Here's how the part is built. I have some questions about the finished solid (model axes, mm). A direction names the side the tool comes from. Round coordinates to 2 decimals unless told otherwise and drop trailing zeros. Loops run counter-clockwise (first coordinate to the right, second up) from the corner with the lowest first, then second, coordinate; pieces in that order, holes last. Notation, with made-up numbers: (85, 16) - (126, 16) arc R17 ccw to (126, 49) - close; hole circle Ø5 at (-21, -28.5). An arc over 180 degrees is marked (long way). Answer as a JSON object with one key per item and string values. Group by question number.
1) If I drill on line 1 along X through (y, z) = (43, 50); line 2 along X through (y, z) = (-6, 59.5); line 3 along Y through (x, z) = (5, 32), over which ranges is the centre line in solid material (lowest first)? Write a range as [from, to].
2) I want a section at A-A, the plane z = 32. Please give me the cut outline in (x, y), then the cut area to 3 significant figures.
3) If we mould it in two halves opening along X, with no side actions, what happens to faces 5 (the face through (-25, 38, 32)), 6 (the face through (-50, 2, 63)), 7 (the face through (12.082, 85.524, 27.664))? For each: pulls with the +X half, pulls with the -X half, needs draft (parallel to the pull), parting line crosses it, or undercut.
4) I want a section at D-D, the plane y = 2. Please give me the cut outline in (x, z), then the cut area to 3 significant figures.
5) I want a section at C-C, the plane y = 79. Please give me the cut outline in (x, z), then the cut area to 3 significant figures.
6) Which directions (+Z, -Z, +X, -X, +Y, -Y) give clear straight access to the entire face, cutting with the end or side of a thin tool? Please do faces 1 (the face through (37, 24, 30)), 2 (the face through (-57.098, 27.468, 58.084)), 3 (the face through (28, 21, 35)), 4 (the face through (-37, -6, 32)).
7) I want a section at B-B, the plane x = 6. Please give me the cut outline in (y, z), then the cut area to 3 significant figures.
8) Will these pins go through, and if not, where does the flat tip stop? P1, Ø8, axis at x = 4.5, z = 39, coming from the -Y side; P2, Ø10, axis at x = 9.5, y = 66.5, coming from the +Z side; P3, Ø15.5, axis at x = -15.74, z = 49.83, coming from the +Y side.
from build123d import *

# Parameters (mm, degrees)
BASE_PROFILE_SKETCH_W           = 128
BASE_PROFILE_SKETCH_H           = 20
BASE_PLATE_DEPTH                = 64
UNDERSIDE_RELIEF_CUT_DEPTH      = 92.060419503
UNDERSIDE_RELIEF_CUT_DEPTH_BACK = 64
UNDERSIDE_RELIEF_SKETCH_W       = 55
UNDERSIDE_RELIEF_SKETCH_H       = 8
FIRST_UPRIGHT_SKETCH_W          = 14
FIRST_UPRIGHT_SKETCH_H          = 64
FIRST_UPRIGHT_DEPTH             = 56
FIRST_TRUNNION_BOSS_DEPTH       = 10
FIRST_TRUNNION_BOSS_DEPTH_BACK  = 14
FIRST_TRUNNION_BOSS_SKETCH_R    = 20
FIRST_TRUNNION_BOSS_SKETCH_R_2  = 10
FIRST_TRUNNION_BORE_DEPTH       = 14
FIRST_UPRIGHT_TAPER_CUT_DEPTH   = 14
CENTER_BLOCK_DEPTH              = 28
SECOND_TRUNNION_BOSS_SKETCH_R   = 20
SECOND_TRUNNION_BOSS_SKETCH_R_2 = 10
SECOND_TRUNNION_BOSS_DEPTH      = 20
SECOND_UPRIGHT_DEPTH            = 10
SECOND_TRUNNION_BORE_DEPTH      = 10
GUSSET_RIB_REACH                = 120.44
GUSSET_RIB_SKETCH_WALL_W        = 299.707341614
GUSSET_RIB_SKETCH_WALL_H        = 10
BASE_MOUNTING_HOLES_SKETCH_R    = 6
BASE_MOUNTING_HOLES_DEPTH       = 124.887045328


with BuildPart() as part:
    # Base Profile Sketch → Base Plate (new body)
    with BuildSketch(Plane.XY):
        Rectangle(BASE_PROFILE_SKETCH_W, BASE_PROFILE_SKETCH_H)
    extrude(amount=BASE_PLATE_DEPTH)

    # Underside Relief Sketch → Underside Relief Cut (cut, two sides: drawn at the far end of the back side and taken through both)
    with BuildSketch(Plane.XY.offset(-UNDERSIDE_RELIEF_CUT_DEPTH_BACK)):
        with Locations((-9.5, -6)):
            Rectangle(UNDERSIDE_RELIEF_SKETCH_W, UNDERSIDE_RELIEF_SKETCH_H)
    extrude(amount=UNDERSIDE_RELIEF_CUT_DEPTH + UNDERSIDE_RELIEF_CUT_DEPTH_BACK, mode=Mode.SUBTRACT)

    # First Upright Sketch → First Upright (add)
    with BuildSketch(Plane(origin=(0, 10, 0), x_dir=(1, 0, 0), z_dir=(0, 1, 0))):
        with Locations((-57, -32)):
            Rectangle(FIRST_UPRIGHT_SKETCH_W, FIRST_UPRIGHT_SKETCH_H)
    extrude(amount=FIRST_UPRIGHT_DEPTH)

    # First Trunnion Boss Sketch → First Trunnion Boss (add, two sides: drawn at the far end of the back side and taken through both)
    with BuildSketch(Plane.ZY.offset(64).offset(-FIRST_TRUNNION_BOSS_DEPTH_BACK)):
        with Locations((32, 66)):
            Circle(FIRST_TRUNNION_BOSS_SKETCH_R)
        with Locations((32, 66)):
            Circle(FIRST_TRUNNION_BOSS_SKETCH_R_2, mode=Mode.SUBTRACT)
    extrude(amount=FIRST_TRUNNION_BOSS_DEPTH + FIRST_TRUNNION_BOSS_DEPTH_BACK)

    # First Trunnion Bore Sketch → First Trunnion Bore (cut)
    with BuildSketch(Plane.ZY.offset(64)):
        with BuildLine():
            Line((42, 66), (22, 66))
            ThreePointArc((22, 66), (32, 56), (42, 66))
        make_face()
    extrude(amount=-FIRST_TRUNNION_BORE_DEPTH, mode=Mode.SUBTRACT)

    # First Upright Taper Sketch → First Upright Taper Cut (cut)
    with BuildSketch(Plane.ZY.offset(64)):
        Polygon((12, 66), (0, -10), (0, 66), align=None)
        Polygon((64, -10), (52, 66), (64, 66), align=None)
    extrude(amount=-FIRST_UPRIGHT_TAPER_CUT_DEPTH, mode=Mode.SUBTRACT)

    # Center Block Sketch → Center Block (add)
    with BuildSketch(Plane(origin=(0, 10, 0), x_dir=(1, 0, 0), z_dir=(0, 1, 0))):
        Polygon((-50, -32), (-50, -26), (0, -26), (0, -38), (-50, -38), align=None)
    extrude(amount=CENTER_BLOCK_DEPTH)



with BuildPart() as body_2:
    # Second Trunnion Boss Sketch → Second Trunnion Boss (new body)
    with BuildSketch(Plane(origin=(0, 0, 0), x_dir=(0, 0, -1), z_dir=(1, 0, 0))):
        with Locations(Location((-32, 66, 0), (0, 0, 180))):
            Circle(SECOND_TRUNNION_BOSS_SKETCH_R)
        with Locations(Location((-32, 66, 0), (0, 0, 180))):
            Circle(SECOND_TRUNNION_BOSS_SKETCH_R_2, mode=Mode.SUBTRACT)
    extrude(amount=SECOND_TRUNNION_BOSS_DEPTH)


with BuildPart() as part_1:
    add(part.part)

    add(body_2.part)  # Second Upright merges body 2
    # Second Upright Sketch → Second Upright (add)
    with BuildSketch(Plane(origin=(0, 0, 0), x_dir=(0, 0, -1), z_dir=(1, 0, 0))):
        Polygon((-52, 66), (-60.842105263, 10), (-3.157894737, 10), (-12, 66), align=None)
    extrude(amount=SECOND_UPRIGHT_DEPTH)

    # Second Trunnion Bore Sketch → Second Trunnion Bore (cut)
    with BuildSketch(Plane(origin=(0, 0, 0), x_dir=(0, 0, -1), z_dir=(1, 0, 0))):
        with BuildLine():
            Line((-22, 66), (-42, 66))
            ThreePointArc((-42, 66), (-32, 56), (-22, 66))
        make_face()
    extrude(amount=SECOND_TRUNNION_BORE_DEPTH, mode=Mode.SUBTRACT)

    # Gusset Rib Sketch wall → Gusset Rib (add, up to next)
    with BuildSketch(Plane(origin=(37, 24, 30), x_dir=(0.887754531449, -0.460317164455, 0), z_dir=(0.460317164455, 0.887754531449, 0)), mode=Mode.PRIVATE) as gusset_rib_sk1:
        Rectangle(GUSSET_RIB_SKETCH_WALL_W, GUSSET_RIB_SKETCH_WALL_H)
    gusset_rib_tool1 = extrude(gusset_rib_sk1.sketch, amount=-GUSSET_RIB_REACH, mode=Mode.PRIVATE) - part_1.part
    add(gusset_rib_tool1.solids().sort_by_distance((37, 24, 30))[0])

    # Base Mounting Holes Sketch → Base Mounting Holes (cut, through all)
    with BuildSketch(Plane(origin=(0, 10, 0), x_dir=(1, 0, 0), z_dir=(0, 1, 0))):
        with Locations(Location((-15.743786959, -13.828319493, 0), (0, 0, 180))):
            Circle(BASE_MOUNTING_HOLES_SKETCH_R)
        with Locations(Location((-15.743786959, -49.828319493, 0), (0, 0, 180))):
            Circle(BASE_MOUNTING_HOLES_SKETCH_R)
        with Locations(Location((44.704140343, -13.828319493, 0), (0, 0, 180))):
            Circle(BASE_MOUNTING_HOLES_SKETCH_R)
        with Locations(Location((44.704140343, -49.828319493, 0), (0, 0, 180))):
            Circle(BASE_MOUNTING_HOLES_SKETCH_R)
    extrude(amount=-BASE_MOUNTING_HOLES_DEPTH, mode=Mode.SUBTRACT)


solid = part_1.part
Outcome:
{
 "1": {"line 1": "[-64, -50], [0, 10]", "line 2": "[-64, -37], [18, 64]", "line 3": "[-2, 56], [76, 86]"},
 "2": {"outline": "(-74, 46) - (-64, 46) - (-64, -10) - (-37, -10) - (-37, -2) - (18, -2) - (18, -10) - (64, -10) - (64, 10) - (10, 38) - (10, 46) - (20, 46) - (20, 56) - (0, 56) - (0, 38) - (-50, 38) - (-50, 56) - (-74, 56) - close; (-74, 76) - (-50, 76) - (-50, 86) - (-74, 86) - close; (0, 76) - (20, 76) - (20, 86) - (0, 86) - close", "area": "6,020 mm^2"},
 "3": {"face 5": "undercut", "face 6": "pulls with the -X half", "face 7": "needs draft"},
 "4": {"outline": "(-64, 1.89) - (-50, 1.89) - (-50, 0) - (64, 0) - (64, 64) - (-50, 64) - (-50, 62.11) - (-64, 62.11) - close; hole circle Ø12 at (-15.74, 13.83); hole circle Ø12 at (-15.74, 49.83); hole circle Ø12 at (44.7, 13.83); hole circle Ø12 at (44.7, 49.83)", "area": "7,690 mm^2"},
 "5": {"outline": "(-74, 16.8) - (-50, 16.8) - (-50, 47.2) - (-74, 47.2) - close; (0, 16.8) - (20, 16.8) - (20, 47.2) - (0, 47.2) - close", "area": "1,340 mm^2"},
 "6": {"face 1": "+Z, -Z, +X", "face 2": "+Z, -X, +Y", "face 3": "+Z, +X", "face 4": "+Z, -Z, -Y"},
 "7": {"outline": "(-2, 0) - (10, 0) - (10, 3.16) - (66, 12) arc R20 ccw to (66, 52) - (10, 60.84) - (10, 64) - (-2, 64) - close; hole circle Ø20 at (66, 32)", "area": "3,820 mm^2"},
 "8": {"P1": "y = -2", "P2": "z = 52.71", "P3": "y = 10"}
}
